Input: part model. Units: mm. Frame: model coordinates. A direction names the side the tool comes from. Coordinates: 2 decimals unless noted, no trailing zeros. Order: outer loops, then holes, each group sorted by start corner. A loop starts at its lowest first (then second) coordinate and runs counter-clockwise, first axis right, second up. Notation, with made-up numbers: M 45.25,32.25 L 78.25,32.25 A28 ccw 78.25,67.25 Z; hole C -31,44 d6. An arc over 180 degrees is marked long. Answer in a Markdown table with one row per item.
from build123d import *

# Parameters (mm, degrees)
SKETCH1_W               = 5
SKETCH1_H               = 5
BOSS_EXTRUDE1_DEPTH     = 270
SKETCH2_W               = 10
SKETCH2_H               = 5
BOSS_EXTRUDE2_DEPTH     = 18
SKETCH3_W               = 5
SKETCH3_H               = 19.358131828
CUT_EXTRUDE1_DEPTH      = 12
CUT_EXTRUDE2_DEPTH      = 289.18440277
CUT_EXTRUDE2_DEPTH_BACK = 289.18440277
SKETCH4_R               = 1
SKETCH5_W               = 5
SKETCH5_H               = 5
BOSS_EXTRUDE3_DEPTH     = 180


with BuildPart() as part:
    # Sketch1 → Boss-Extrude1 (new body)
    with BuildSketch(Plane.XY):
        Rectangle(SKETCH1_W, SKETCH1_H)
    extrude(amount=BOSS_EXTRUDE1_DEPTH)

    # Sketch2 → Boss-Extrude2 (add)
    with BuildSketch(Plane.XY.offset(270)):
        Rectangle(SKETCH2_W, SKETCH2_H)
    extrude(amount=BOSS_EXTRUDE2_DEPTH)

    # Sketch3 → Cut-Extrude1 (cut)
    with BuildSketch(Plane.XY.offset(288)):
        Rectangle(SKETCH3_W, SKETCH3_H)
    extrude(amount=-CUT_EXTRUDE1_DEPTH, mode=Mode.SUBTRACT)

    # Sketch4 → Cut-Extrude2 (cut, two sides: drawn at the far end of the back side and taken through both)
    with BuildSketch(Plane(origin=(5, 0, 0), x_dir=(0, 0, -1), z_dir=(1, 0, 0)).offset(-CUT_EXTRUDE2_DEPTH_BACK)):
        with Locations(Location((-280.07674021, 0, 0), (0, 0, 90))):
            Circle(SKETCH4_R)
        with BuildLine():
            Line((-280.07674021, 2.5), (-280.07674021, 12.098504892))
            Line((-280.07674021, 12.098504892), (-285.8811548, 12.098504892))
            Line((-285.8811548, 12.098504892), (-318.827178265, -19.142217328))
            Line((-318.827178265, -19.142217328), (-280.07674021, -2.5))
            ThreePointArc((-280.07674021, -2.5), (-282.57674021, 0), (-280.07674021, 2.5))
        make_face()
    extrude(amount=CUT_EXTRUDE2_DEPTH + CUT_EXTRUDE2_DEPTH_BACK, mode=Mode.SUBTRACT)

    # Sketch5 → Boss-Extrude3 (add)
    with BuildSketch(Plane(origin=(0, 0, 0), x_dir=(1, 0, 0), z_dir=(0, 1, 0))):
        with Locations((0, -116)):
            Rectangle(SKETCH5_W, SKETCH5_H)
    extrude(amount=BOSS_EXTRUDE3_DEPTH)


solid = part.part
1) Cut plane B-B, the plane z = 121.5. Output: boundary loops of the cut face in (x, y), and give its area (3 significant figures).
Resolved:
| item | result |
|---|---|
| outline | M -2.5,-2.5 L 2.5,-2.5 L 2.5,2.5 L -2.5,2.5 Z |
| area | 25.0 mm2 |
2) Reachability of faces 1 (the face through (0, 2.5, 198)), 2 (the face through (2.5, 48, 116)), 3 (the face through (-2.5, 48, 114)), 4 (the face through (0, -2.5, 138)) from +Z, -Z, +X, -X, +Y, -Y: full face, straight path, thin tool, end or side. Return the list, or none.
Resolved:
| item | result |
|---|---|
| face 1 | +Z, +X, -X, +Y |
| face 2 | -Z, +X, +Y, -Y |
| face 3 | -Z, -X, +Y, -Y |
| face 4 | +Z, -Z, +X, -X, -Y |
3) Cut plane C-C, the plane y = 99. Output: boundary loops of the cut face in (x, z), and give its area (3 significant figures).
Resolved:
| item | result |
|---|---|
| outline | M -2.5,113.5 L 2.5,113.5 L 2.5,118.5 L -2.5,118.5 Z |
| area | 25.0 mm2 |
4) Cut plane A-A, the plane x = -0.5. Output: boundary loops of the cut face in (y, z).
Resolved:
| item | result |
|---|---|
| outline | M -2.5,0 L 2.5,0 L 2.5,113.5 L 180,113.5 L 180,118.5 L 2.5,118.5 L 2.5,276 L -2.5,276 Z |
5) Material intervals for probe 1 along Z at (x, y) = (4.4, 0); probe 2 along Y at (x, z) = (1.5, 72); probe 3 along Z at (x, y) = (-1.75, 136), sorted ascending.
Resolved:
| item | result |
|---|---|
| probe 1 | z = 270 to 279.08, 281.08 to 282.58 |
| probe 2 | y = -2.5 to 2.5 |
| probe 3 | z = 113.5 to 118.5 |
6) Contact query for flat-ended pins moving along their axis: pin 1 (6 mm diameter, centred on x = 0.5, y = 50, fed in from -Z); pin 2 (1.2 mm diameter, centred on x = -3.5, y = -1, fed in from -Z); pin 3 (1 mm diameter, centred on x = -4, z = 90, fed in from +Y); pin 4 (2.5 mm diameter, centred on x = 0, z = 36, fed in from +Y). Output: stop coordinate, or through.
Resolved:
| item | result |
|---|---|
| pin 1 | stops at z = 113.5 |
| pin 2 | stops at z = 270 |
| pin 3 | passes through |
| pin 4 | stops at y = 2.5 |
